```python
from build123d import *

# Parameters (mm, degrees)
SKETCH_1_W         = 21
SKETCH_1_H         = 6
EXTRUDE_1_DEPTH    = 6
HOLE_WIZARD_M3_1_D = 2.5
HOLE_WIZARD_M3_2_D = 2.5


with BuildPart() as part:
    # 草图1 → 凸台-拉伸1 (new body)
    with BuildSketch(Plane(origin=(0, 0, 0), x_dir=(1, 0, 0), z_dir=(0, 1, 0))):
        Rectangle(SKETCH_1_W, SKETCH_1_H)
    extrude(amount=EXTRUDE_1_DEPTH)

    # M3 螺纹孔1 (through all)
    with Locations(Plane.XY.offset(3)):
        with Locations((-2.5, 3), (7.5, 3)):
            Hole(HOLE_WIZARD_M3_1_D / 2)

    # M3 螺纹孔2 (through all)
    with Locations(Plane(origin=(0, 6, 0), x_dir=(1, 0, 0), z_dir=(0, 1, 0))):
        with Locations((2.5, 0), (-7.5, 0)):
            Hole(HOLE_WIZARD_M3_2_D / 2)


solid = part.part
```
For this review, take the finished solid that the model builds, in its own axes (mm). Coordinates: 2 decimals unless noted, no trailing zeros. Loops run counter-clockwise (first coordinate to the right, second up) from the corner with the lowest first, then second, coordinate; pieces in that order, holes last.
1. Add section C-C, the plane x = -2.5. Give the boundary of the cut face in (y, z), then the cut area to 3 significant figures.
2. For line 1 (Z direction, x = -7.5, y = 1.55); line 2 (X direction, y = 2.3, z = -0.85); line 3 (X direction, y = 1, z = -0.5), list the stretches that pass through material, from the lowest coordinate up.
3. Add section A-A, the plane z = 0. Give the boundary of the cut face in (x, y).
4. Mouldability with a two-part tool opening along Z and no side actions: class faces 1 (the flat face through (0, 3, 3)), 2 (the cylindrical face through (1.31, 2.96, -0.38)), 3 (the cylindrical face through (8.421, 3.845, -0.042)), 4 (the flat face through (0, 3, -3)) as +Z half, -Z half, draft (parallel to the pull), parting line (faces both ways), or undercut.
5. Add section D-D, the plane y = 1.1. Give the boundary of the cut face in (x, z).
6. Add section B-B, the plane y = 3.75. Give the boundary of the cut face in (x, z), then the cut area to 3 significant figures.
7. Insertion check: P1, Ø1.5, axis at x = -7.5, z = 0, coming from the +Y side. The pin has a flat end and moves straight along its axis. Give the tip position at first contact, or say it passes through.
Result:
1. outline: (0, -3) - (1.75, -3) - (1.75, 3) - (0, 3) - close; (4.25, -3) - (6, -3) - (6, 3) - (4.25, 3) - close
1. area: 21.0 mm2
2. line 1: z = -3 to -1.25, 1.25 to 3
2. line 2: x = -10.5 to -8.42, -6.58 to -3.54, -1.46 to 1.58, 3.42 to 6.46, 8.54 to 10.5
2. line 3: x = -10.5 to -8.65, -6.35 to 1.35, 3.65 to 10.5
3. outline: (-10.5, 0) - (-8.75, 0) - (-8.75, 6) - (-10.5, 6) - close; (-6.25, 0) - (1.25, 0) - (1.25, 6) - (-6.25, 6) - close; (3.75, 0) - (10.5, 0) - (10.5, 6) - (3.75, 6) - close; hole circle Ø2.5 at (-2.5, 3); hole circle Ø2.5 at (7.5, 3)
4. face 1: +Z half
4. face 2: undercut
4. face 3: draft
4. face 4: -Z half
5. outline: (-10.5, -3) - (10.5, -3) - (10.5, 3) - (-10.5, 3) - close; hole circle Ø2.5 at (-7.5, 0); hole circle Ø2.5 at (2.5, 0)
6. outline: (-10.5, -3) - (-3.5, -3) - (-3.5, 3) - (-10.5, 3) - close; (-1.5, -3) - (6.5, -3) - (6.5, 3) - (-1.5, 3) - close; (8.5, -3) - (10.5, -3) - (10.5, 3) - (8.5, 3) - close; hole circle Ø2.5 at (-7.5, 0); hole circle Ø2.5 at (2.5, 0)
6. area: 92.2 mm2
7. P1: passes through
